```python
from build123d import *

# Parameters (mm, degrees)
SKETCH_1_W             = 15
SKETCH_1_H             = 12.5
EXTRUDE_1_DEPTH        = 450
SKETCH_2_R             = 3
CUT_EXTRUDE_1_DEPTH    = 4.5
SKETCH_3_R             = 2.25
CUT_EXTRUDE_2_DEPTH    = 451.236049201
PATTERN_LINEAR_1_COUNT = 16
PATTERN_LINEAR_1_PITCH = 60


with BuildPart() as part:
    # 草图1 → 凸台-拉伸1 (new, symmetric)
    with BuildSketch(Plane.XY):
        Rectangle(SKETCH_1_W, SKETCH_1_H)
    extrude(amount=EXTRUDE_1_DEPTH, both=True)

    # 草图2 → 切除-拉伸1 (cut)
    with BuildSketch(Plane(origin=(0, 6.25, 0), x_dir=(1, 0, 0), z_dir=(0, 1, 0))):
        with Locations(Location((0, -420, 0), (0, 0, 270))):
            Circle(SKETCH_2_R)
    cut_extrude_1 = extrude(amount=-CUT_EXTRUDE_1_DEPTH, mode=Mode.SUBTRACT)

    # 草图3 → 切除-拉伸2 (cut, through all)
    with BuildSketch(Plane(origin=(0, 6.25, 0), x_dir=(1, 0, 0), z_dir=(0, 1, 0))):
        with Locations(Location((0, -420, 0), (0, 0, 270))):
            Circle(SKETCH_3_R)
    cut_extrude_2 = extrude(amount=-CUT_EXTRUDE_2_DEPTH, mode=Mode.SUBTRACT)

    # 阵列(线性)1: 切除-拉伸1, 切除-拉伸2 ×16
    with Locations(*[(0, 0, -i * PATTERN_LINEAR_1_PITCH) for i in range(1, PATTERN_LINEAR_1_COUNT)]):
        add(cut_extrude_1, mode=Mode.SUBTRACT)
        add(cut_extrude_2, mode=Mode.SUBTRACT)


solid = part.part
```
Input: part model. Units: mm. Frame: model coordinates. Give positions to 0.01 mm unless a question says otherwise; leave off trailing zeros. Write item = value, one per line. Start each with the question number.
1) Cut plane A-A (y = -2.25). Give the number of separate pieces and of enclosed holes in the cut face, and give its area (3 significant figures).
2) Pin query (flat end, axial travel): pin 1 (1.8 mm diameter, centred on x = -1.5, z = 121, fed in from +Y). Return the tip coordinate at first contact, or that it passes through.
3) Material intervals for L1, parallel to X at y = 3.1, z = 120; L2, parallel to X at y = 0.25, z = 360, sorted ascending. Write a range as [from, to].
Answers follow:
q1.separate_pieces = 1
q1.enclosed_holes = 15
q1.area = 13,300 mm^2
q2.pin_1 = 1.75
q3.L1 = [-7.5, -3], [3, 7.5]
q3.L2 = [-7.5, -2.25], [2.25, 7.5]
